The listing builds one solid part. Answer for the finished solid, in the listing's coordinates (mm). A direction names the side the tool comes from. Give positions to 0.01 mm unless a question says otherwise; leave off trailing zeros. Loops run counter-clockwise (first coordinate to the right, second up) from the corner with the lowest first, then second, coordinate; pieces in that order, holes last. Notation, with made-up numbers: (33.5, -10.75) - (62.5, -10.75) arc R27 cw to (62.5, 26.25) - close; hole circle Ø3 at (49, 41). An arc over 180 degrees is marked (long way). Write item = value, one per line. Start each with the question number.
1) Flat-ended cylindrical pins translate along their axes: P1, Ø1, axis at x = 21, z = 63, coming from the +Y side; P2, Ø4, axis at y = -41.5, z = 219, coming from the +X side; P3, Ø10, axis at x = 18, z = 169, coming from the -Y side. Find the tip coordinate at first contact, or state that the pin passes through.
2) The part is cut by section C-C on x = 15. Write down the section's boundary in (y, z).
3) The part is cut by section B-B on y = -216. Write down the section's boundary in (x, z), plus the area to 3 significant figures.
4) Consider probe 1 along X at (y, z) = (-117, 127); probe 2 along X at (y, z) = (-30, 168); probe 3 along Y at (x, z) = (5, 157.5). Determine where each line is inside the solid, lowest interval first.
5) The part is cut by section A-A on z = 75. Write down the section's boundary in (x, y), plus the area to 3 significant figures.
6) The part is cut by section D-D on z = 227.5. Write down the section's boundary in (x, y).
7) Which of the six approach directions +Z, -Z, +X, -X, +Y, -Y give full straight-line access (tool end or side, diameter ignored) to faces 1 (the flat face through (40, -198, 133)), 2 (the flat face through (0, -25, 133)), 3 (the flat face through (3, -25, 133))?
from build123d import *

# Parameters (mm, degrees)
EXTRUDE_1_DEPTH     = 270
CUT_EXTRUDE_2_DEPTH = 270


with BuildPart() as part:
    # 草图1 → 凸台-拉伸1 (new body)
    with BuildSketch(Plane.XY):
        Polygon((0, 0), (0, -50), (40, -90), (40, -310), (43, -310), (43, -88.757359313), (3, -48.757359313), (3, 0), align=None)
    extrude(amount=EXTRUDE_1_DEPTH)

    # 草图2 → 切除-拉伸2 (cut)
    with BuildSketch(Plane(origin=(43, 0, 0), x_dir=(0, 0, -1), z_dir=(1, 0, 0))):
        Polygon((-270, 0), (-220, 0), (-270, -88.757359313), align=None)
        Polygon((0, 0), (-50, 0), (0, -88.757359313), align=None)
    extrude(amount=-CUT_EXTRUDE_2_DEPTH, mode=Mode.SUBTRACT)


solid = part.part
Answer below:
q1.P1 = -66.26
q1.P2 = 3
q1.P3 = -73
q2.outline = (-65, 13.38) - (-60.76, 15.77) - (-60.76, 254.23) - (-65, 256.62) - close
q3.outline = (40, 0) - (43, 0) - (43, 270) - (40, 270) - close
q3.area = 810 mm2
q4.probe_1 = 40 to 43
q4.probe_2 = 0 to 3
q4.probe_3 = -55 to -50.76
q5.outline = (0, -50) - (40, -90) - (40, -310) - (43, -310) - (43, -88.76) - (3, -48.76) - (3, 0) - (0, 0) - close
q5.area = 980 mm2
q6.outline = (0, -50) - (40, -90) - (40, -310) - (43, -310) - (43, -88.76) - (3, -48.76) - (3, -13.31) - (0, -13.31) - close
q7.face_1 = +Z, -Z, -X, -Y
q7.face_2 = +Z, -Z, -X, +Y, -Y
q7.face_3 = +Z, -Z, +X, +Y
